from build123d import *

# Parameters (mm, degrees)
SKETCH_1_R      = 6
EXTRUDE_1_DEPTH = 6


with BuildPart() as part:
    # 草图1 → 凸台-拉伸1 (new body)
    with BuildSketch(Plane.XY):
        with BuildLine():
            Line((-42.5, 22.5), (42.5, 22.5))
            Line((42.5, 22.5), (42.5, -14.5))
            ThreePointArc((42.5, -14.5), (40.156854249, -20.156854249), (34.5, -22.5))
            Line((34.5, -22.5), (-34.5, -22.5))
            ThreePointArc((-34.5, -22.5), (-40.156854249, -20.156854249), (-42.5, -14.5))
            Line((-42.5, -14.5), (-42.5, 22.5))
        make_face()
        with Locations((0, 2.5)):
            Circle(SKETCH_1_R, mode=Mode.SUBTRACT)
    extrude(amount=EXTRUDE_1_DEPTH)


solid = part.part
Can you work these out from the model? Positions are in its coordinate system, mm. Coordinates: 2 decimals unless noted, no trailing zeros. Loops run counter-clockwise (first coordinate to the right, second up) from the corner with the lowest first, then second, coordinate; pieces in that order, holes last. Notation, with made-up numbers: (75, -35) - (90, -35) arc R16 cw to (90, -5) - close; hole circle Ø9 at (86, -32). An arc over 180 degrees is marked (long way). Answer as a JSON object with one key per item and string values. Group by question number.
Item 1: If we section it at A-A (y = 2.5): List the corners of the cut face in (x, z) for me, plus the area to 3 significant figures.
Item 2: If we section it at C-C (z = 5): List the corners of the cut face in (x, y) for me.
Item 3: If I drill on L1, parallel to Y at x = 0, z = 4.2; L2, parallel to X at y = -16, z = 1.1; L3, parallel to Y at x = 4.5, z = 2.85, over which ranges is the centre line in solid material (lowest first)? Write a range as from..to.
Item 4: If we section it at B-B (x = 0): List the corners of the cut face in (y, z) for me, plus the area to 3 significant figures.
Item 5: If we mould it in two halves opening along Y, with no side actions, what happens to faces 1 (the face through (-5.994, 2.764, 2.958)), 2 (the face through (0, -22.5, 3)), 3 (the face through (1, -5, 6))? For each: released by +Y, released by -Y, zero draft, split by the parting line, or undercut.
Returned:
{
 "1": {"outline": "(-42.5, 0) - (-6, 0) - (-6, 6) - (-42.5, 6) - close; (6, 0) - (42.5, 0) - (42.5, 6) - (6, 6) - close", "area": "438 mm²"},
 "2": {"outline": "(-42.5, -14.5) arc R8 ccw to (-34.5, -22.5) - (34.5, -22.5) arc R8 ccw to (42.5, -14.5) - (42.5, 22.5) - (-42.5, 22.5) - close; hole circle Ø12 at (0, 2.5)"},
 "3": {"L1": "y = -22.5..-3.5, 8.5..22.5", "L2": "x = -42.36..42.36", "L3": "y = -22.5..-1.47, 6.47..22.5"},
 "4": {"outline": "(-22.5, 0) - (-3.5, 0) - (-3.5, 6) - (-22.5, 6) - close; (8.5, 0) - (22.5, 0) - (22.5, 6) - (8.5, 6) - close", "area": "198 mm²"},
 "5": {"face 1": "undercut", "face 2": "released by -Y", "face 3": "zero draft"}
}
